Verification items for the finished model (mm, model axes). Give positions to 0.01 mm unless a question says otherwise; leave off trailing zeros. Loops run counter-clockwise (first coordinate to the right, second up) from the corner with the lowest first, then second, coordinate; pieces in that order, holes last. Notation, with made-up numbers: (-14.5, 86.25) - (5.5, 86.25) arc R16 ccw to (5.5, 115.25) - close; hole circle Ø5 at (-33, 80.25). An arc over 180 degrees is marked (long way). One line per item, written item: value. Start each with the question number.
1. Sectioned sample at D-D (z = 2.75). Record the cut outline in (x, y), plus the area to 3 significant figures.
2. Sectioned sample at C-C (y = 3.5). Record the cut outline in (x, z), plus the area to 3 significant figures.
3. Gauge pin test, flat ends, axial feed: pin 1 (2 mm diameter, centred on x = 12.5, z = 2, fed in from +Y); pin 2 (2 mm diameter, centred on x = 3, z = 0.5, fed in from +Y); pin 3 (1 mm diameter, centred on y = 6, z = -2.5, fed in from +X). Record the tip position at first contact, or that the pin passes through.
4. Scan lines: L1, parallel to Y at x = 14.5, z = 1; L2, parallel to X at y = 5.5, z = 2.25; L3, parallel to Y at x = 7.25, z = 1.5. Record each from-to range of solid material in increasing order. Write a range as [from, to].
5. Mould release check, pull along X, two halves, no side actions. Record for faces 1 (the flat face through (7, 1, 0)), 2 (the flat face through (0, 0.5, 0)), 3 (the cylindrical face through (12, 3.6, 0)): pulls with the +X half, pulls with the -X half, needs draft (parallel to the pull), parting line crosses it, or undercut.
6. Sectioned sample at B-B (z = 0). Record the cut outline in (x, y).
7. Sectioned sample at A-A (x = 4.8). Record the cut outline in (y, z).
from build123d import *

# Parameters (mm, degrees)
SKETCH_1_R          = 2.5
EXTRUDE_1_DEPTH     = 3.3
SKETCH_2_R          = 1.65
CUT_EXTRUDE_1_DEPTH = 6.6


with BuildPart() as part:
    # 草图1 → 凸台-拉伸1 (new, symmetric)
    with BuildSketch(Plane.XY):
        with BuildLine():
            Line((0, 1), (0, 0))
            Line((0, 0), (14.5, 0))
            ThreePointArc((14.5, 0), (15.822875656, 6.740370349), (12.050510257, 1))
            Line((12.050510257, 1), (0, 1))
        make_face()
        with Locations((14.5, 3.5)):
            Circle(SKETCH_1_R, mode=Mode.SUBTRACT)
    extrude(amount=EXTRUDE_1_DEPTH, both=True)

    # 草图2 → 切除-拉伸1 (cut)
    with BuildSketch(Plane(origin=(0, 1, 0), x_dir=(1, 0, 0), z_dir=(0, 1, 0))):
        with Locations(Location((4.8, 0, 0), (0, 0, 270))):
            Circle(SKETCH_2_R)
    extrude(amount=-CUT_EXTRUDE_1_DEPTH, mode=Mode.SUBTRACT)


solid = part.part
Results are:
1. outline: (0, 0) - (14.5, 0) arc R3.5 ccw (long way) to (12.05, 1) - (0, 1) - close; hole circle Ø5 at (14.5, 3.5)
1. area: 31.7 mm^2
2. outline: (11, -3.3) - (12, -3.3) - (12, 3.3) - (11, 3.3) - close; (17, -3.3) - (18, -3.3) - (18, 3.3) - (17, 3.3) - close
2. area: 13.2 mm^2
3. pin 1: stops at y = 6.85
3. pin 2: stops at y = 1
3. pin 3: stops at x = 17.37
4. L1: y = [0, 1], [6, 7]
4. L2: x = [11.63, 13], [16, 17.37]
4. L3: y = [0, 1]
5. face 1: needs draft
5. face 2: pulls with the -X half
5. face 3: undercut
6. outline: (0, 0) - (3.15, 0) - (3.15, 1) - (0, 1) - close; (6.45, 0) - (14.5, 0) arc R3.5 ccw (long way) to (12.05, 1) - (6.45, 1) - close; hole circle Ø5 at (14.5, 3.5)
7. outline: (0, -3.3) - (1, -3.3) - (1, -1.65) - (0, -1.65) - close; (0, 1.65) - (1, 1.65) - (1, 3.3) - (0, 3.3) - close
